Can you work these out from the model? Positions are in its coordinate system, mm. Face numbers are marked on the shaded views. A direction names the side the tool comes from. Give positions to 0.01 mm unless a question says otherwise; leave off trailing zeros. Write each loop counter-clockwise with the first axis right and the second up, starting at its lowest first coordinate (ties: lowest second). Pieces come first, ordered by that corner, then holes.
1. Suppose I cut it at D-D (x = 40.5). Please give me the cut outline in (y, z), and give its area (3 significant figures).
2. If I drill on probe 1 along Y at (x, z) = (19.5, 0); probe 2 along Y at (x, z) = (11.5, 5); probe 3 along Z at (x, y) = (18, 3.25), over which ranges is the centre line in solid material (lowest first)?
3. On a 3-axis mill with a long thin cutter (end or side, diameter ignored), from which of +Z, -Z, +X, -X, +Y, -Y can I reach the whole of each face in a straight line? I mean the marked faces 1 and 2. Say none if no direction works.
4. Thinking about a two-plate mould opening in Z: for the marked faces 3 and 4, which applies, pulls with the +Z half, pulls with the -Z half, needs draft (parallel to the pull), parting line crosses it, or undercut?
5. Suppose I cut it at A-A (y = 0). Please give me the cut outline in (x, z).
6. I'm going to push flat-ended pins straight in: pin 1 (10 mm diameter, centred on y = 0, z = 0, fed in from +X); pin 2 (4 mm diameter, centred on x = 18.5, z = -2.5, fed in from +Y); pin 3 (1 mm diameter, centred on x = 28, y = 4, fed in from -Z); pin 4 (1 mm diameter, centred on x = 19, y = 7.5, fed in from +Z). Where does each tip first touch, or does it pass through?
7. Suppose I cut it at C-C (x = 11). Please give me the cut outline in (y, z), and give its area (3 significant figures).
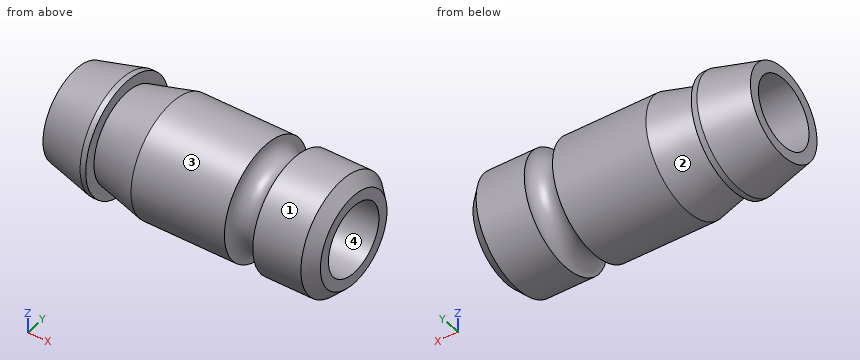
```python
from build123d import *

# Parameters (mm, degrees)
SKETCH2_R          = 6.15
CUT_EXTRUDE1_DEPTH = 99


with BuildPart() as part:
    # Sketch1 → Revolve1 (revolve)
    with BuildSketch(Plane.XY, mode=Mode.PRIVATE) as revolve1_sk:
        with BuildLine():
            Line((17.000000001, 10.1), (9.000000001, 8.100000002))
            Line((9.000000001, 8.100000002), (9.000000001, 10.1))
            Line((9.000000001, 10.1), (8.000000001, 10.1))
            Line((8.000000001, 10.1), (0, 8.100000002))
            Line((0, 8.100000002), (0, 0))
            Line((0, 0), (49, 0))
            Line((49, 0), (49, 8.099999999))
            Line((49, 8.099999999), (46.999999999, 10.1))
            Line((46.999999999, 10.1), (38.500000001, 10.1))
            ThreePointArc((38.500000001, 10.1), (36.000000001, 7.6), (33.500000001, 10.1))
            Line((33.500000001, 10.1), (17.000000001, 10.1))
        make_face()
    revolve(revolve1_sk.sketch.rotate(Axis((0, 0, 0), (1, 0, 0)), 90), axis=Axis((0, 0, 0), (1, 0, 0)))

    # Sketch2 → Cut-Extrude1 (cut)
    with BuildSketch(Plane.ZY):
        Circle(SKETCH2_R)
    extrude(amount=-CUT_EXTRUDE1_DEPTH, mode=Mode.SUBTRACT)


solid = part.part
```
Checks:
1. outline: circle Ø20.2 at (0, 0); hole circle Ø12.3 at (0, 0)
1. area: 202 mm2
2. probe 1: y = -10.1 to -6.15, 6.15 to 10.1
2. probe 2: y = -7.15 to -3.58, 3.58 to 7.15
2. probe 3: z = -9.56 to -5.22, 5.22 to 9.56
3. face 1: +X, -X
3. face 2: none
4. face 3: parting line crosses it
4. face 4: undercut
5. outline: (0, -8.1) - (8, -10.1) - (9, -10.1) - (9, -8.1) - (17, -10.1) - (33.5, -10.1) arc R2.5 cw to (38.5, -10.1) - (47, -10.1) - (49, -8.1) - (49, -6.15) - (0, -6.15) - close; (0, 6.15) - (49, 6.15) - (49, 8.1) - (47, 10.1) - (38.5, 10.1) arc R2.5 cw to (33.5, 10.1) - (17, 10.1) - (9, 8.1) - (9, 10.1) - (8, 10.1) - (0, 8.1) - close
6. pin 1: passes through
6. pin 2: stops at y = 10.09
6. pin 3: stops at z = -9.47
6. pin 4: stops at z = 7.28
7. outline: circle Ø17.2 at (0, 0); hole circle Ø12.3 at (0, 0)
7. area: 114 mm2
